Verification items for this drawing (mm, ordinates from the low corner). A direction names the side the tool comes from. Give positions to 0.01 mm unless a question says otherwise; leave off trailing zeros. Loops run counter-clockwise (first coordinate to the right, second up) from the corner with the lowest first, then second, coordinate; pieces in that order, holes last. Notation, with made-up numbers: (-39, 51) -> (-29, 51) arc R6 cw to (-29, 58) -> close; hole circle Ø4 at (62.25, -34.5). An arc over 180 degrees is marked (long way). Answer as a JSON object with one key per item and string values.
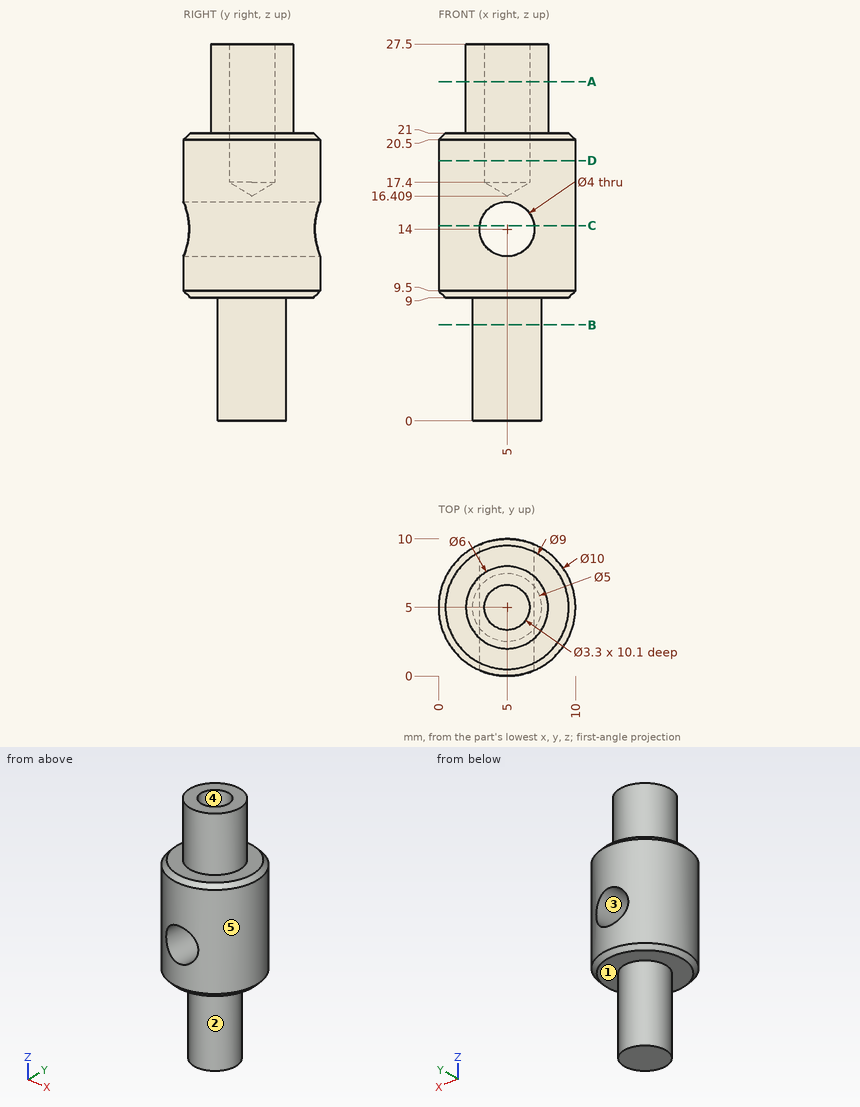
1) Material ranges on line 1 along Y through (x, z) = (5, 25); line 2 along X through (y, z) = (7, 14); line 3 along X through (y, z) = (2.75, 14.75) (1 decimal), recorded low to high. Write a range as from..to.
Geometry check:
{"line 1": "y = 2..3.35, 6.65..8", "line 2": "x = 0.42..3, 7..9.58", "line 3": "x = 0.5..3.1, 6.9..9.5"}
2) Section check D-D on z = 19. Record the cut outline in (x, y).
Geometry check:
{"outline": "circle Ø10 at (5, 5); hole circle Ø3.3 at (5, 5)"}
3) Depth check by flat-ended pin: P1, Ø3.5, axis at x = 5, z = 14, coming from the -Y side; P2, Ø1.5, axis at x = 3, z = 16, coming from the -Y side; P3, Ø1, axis at x = 3, z = 7, coming from the +Y side; P4, Ø3, axis at y = 1, z = 11, coming from the +X side. Enter the tip coordinate at first touch or a pass-through.
Geometry check:
{"P1": "passes through", "P2": "stops at y = 0.16", "P3": "stops at y = 7", "P4": "stops at x = 9.33"}
4) Section check B-B on z = 7. Record the cut outline in (x, y), plus the area to 3 significant figures.
Geometry check:
{"outline": "circle Ø5 at (5, 5)", "area": "19.6 mm2"}
5) Draft check along X on the marked faces 1, 2 and 3. Enter one of: pulls with the +X half, pulls with the -X half, needs draft (parallel to the pull), parting line crosses it, or undercut.
Geometry check:
{"face 1": "needs draft", "face 2": "parting line crosses it", "face 3": "undercut"}
6) Section check C-C on z = 14.25. Record the cut outline in (x, y) (1 decimal).
Geometry check:
{"outline": "(3, 0.4) -> (3, 9.6) arc R5 ccw to start; (7, 0.4) arc R5 ccw to (7, 9.6) -> close"}
7) Section check A-A on z = 24.75. Record the cut outline in (x, y).
Geometry check:
{"outline": "circle Ø6 at (5, 5); hole circle Ø3.3 at (5, 5)"}
8) Tool access check on the marked faces 4 and 5. Record the directions out of +Z, -Z, +X, -X, +Y, -Y that give a thin tool (end or side, any length) a straight path to the whole face; none if there is none.
Geometry check:
{"face 4": "+Z", "face 5": "+Z, -Z"}
